Input: part model. Units: mm. Frame: model coordinates. A direction names the side the tool comes from. Coordinates: 2 decimals unless noted, no trailing zeros. Write each loop counter-clockwise with the first axis right and the second up, starting at its lowest first coordinate (ties: lowest second). Pieces come first, ordered by that corner, then holes. Notation, with made-up numbers: M -8,-38 L 4,-38 A23 cw 4,-20 Z; hole C -13.5,14.5 d4. An arc over 180 degrees is marked long. Use one line per item in the form item = value.
from build123d import *

# Parameters (mm, degrees)
BOSS_EXTRUDE1_DEPTH          = 30
CUT_EXTRUDE1_DEPTH           = 15
F_9_0_9_DIAMETER_HOLE1_D     = 9
F_9_0_9_DIAMETER_HOLE1_DEPTH = 10
F_9_0_9_DIAMETER_HOLE1_TIP   = 2.703872786
M8_TAPPED_HOLE1_D            = 6.8


with BuildPart() as part:
    # Sketch1 → Boss-Extrude1 (new body)
    with BuildSketch(Plane.XY):
        Polygon((0, 0), (0, 10), (17.5, 10), (17.5, 50), (42.5, 50), (42.5, 10), (60, 10), (60, 0), align=None)
    extrude(amount=BOSS_EXTRUDE1_DEPTH)

    # Sketch2 → Cut-Extrude1 (cut)
    with BuildSketch(Plane.XY.offset(30)):
        with BuildLine():
            Line((38.5, 50), (38.5, 35))
            ThreePointArc((38.5, 35), (30, 26.5), (21.5, 35))
            Line((21.5, 35), (21.5, 50))
            ThreePointArc((21.5, 50), (30, 58.5), (38.5, 50))
        make_face()
    extrude(amount=-CUT_EXTRUDE1_DEPTH, mode=Mode.SUBTRACT)

    # Ø9.0 (9) Diameter Hole1
    with Locations(Plane(origin=(7.5, 0, 15), x_dir=(-1, 0, 0), z_dir=(0, -1, 0))):
        with Locations((0, 0), (-45, 0)):
            Hole(F_9_0_9_DIAMETER_HOLE1_D / 2, depth=F_9_0_9_DIAMETER_HOLE1_DEPTH)
            with Locations((0, 0, -(F_9_0_9_DIAMETER_HOLE1_DEPTH + F_9_0_9_DIAMETER_HOLE1_TIP / 2))):  # 118° drill point
                Cone(0, F_9_0_9_DIAMETER_HOLE1_D / 2, F_9_0_9_DIAMETER_HOLE1_TIP, mode=Mode.SUBTRACT)

    # M8 Tapped Hole1 (through all)
    with Locations(Plane(origin=(30, 39, 0), x_dir=(-1, 0, 0), z_dir=(0, 0, -1))):
        with Locations((0, 0)):
            Hole(M8_TAPPED_HOLE1_D / 2)


solid = part.part
(1) Line query: probe 1 along Z at (x, y) = (7.5, 2.75); probe 2 along Y at (x, z) = (30, 10.5); probe 3 along X at (y, z) = (44, 20.75). Output: solid intervals per line, ascending.
Computed:
probe_1 = 0 to 10.5, 19.5 to 30
probe_2 = 0 to 35.6, 42.4 to 50
probe_3 = 17.5 to 21.5, 38.5 to 42.5
(2) Section query B-B on y = 39. Return the cut outline in (x, z).
Computed:
outline = M 17.5,0 L 26.6,0 L 26.6,15 L 21.5,15 L 21.5,30 L 17.5,30 Z; M 33.4,0 L 42.5,0 L 42.5,30 L 38.5,30 L 38.5,15 L 33.4,15 Z
(3) Section query A-A on x = 52.5. Return the cut outline in (y, z).
Computed:
outline = M 0,0 L 10,0 L 10,10.5 L 0,10.5 Z; M 0,19.5 L 10,19.5 L 10,30 L 0,30 Z
(4) Section query D-D on y = 8. Return the cut outline in (x, z), plus the area to 3 significant figures.
Computed:
outline = M 0,0 L 60,0 L 60,30 L 0,30 Z; hole C 7.5,15 d9; hole C 52.5,15 d9
area = 1,670 mm^2
(5) Section query C-C on z = 28.25. Return the cut outline in (x, y), plus the area to 3 significant figures.
Computed:
outline = M 0,0 L 60,0 L 60,10 L 42.5,10 L 42.5,50 L 38.5,50 L 38.5,35 A8.5 cw 21.5,35 L 21.5,50 L 17.5,50 L 17.5,10 L 0,10 Z
area = 1,230 mm^2
(6) Pull-direction query (X, two-part tool) for faces 4 (the flat face through (38.5, 43, 23)), 5 (the flat face through (13, 10, 15)), 6 (the flat face through (17.5, 30, 15)); classes: pulls with the +X half, pulls with the -X half, needs draft (parallel to the pull), parting line crosses it, or undercut.
Computed:
face_4 = undercut
face_5 = needs draft
face_6 = pulls with the -X half
(7) First-contact query: pin 1 Ø13.5 at (x, y) = (28.5, 42.5) entering from +Z; pin 2 Ø14.5 at (x, z) = (7.5, 15) entering from +Y; pin 3 Ø12 at (y, z) = (44.5, 22.5) entering from -X; pin 4 Ø3 at (x, y) = (29.5, 38.5) entering from -Z. Flat tips, straight axial feed; report the tip coordinate or a pass-through.
Computed:
pin_1 = 15
pin_2 = 10
pin_3 = 17.5
pin_4 = through
(8) Set-up query: faces 1 (the flat face through (21.5, 42, 23)), 2 (the cylindrical face through (31.828, 41.867, 7.605)), 3 (the flat face through (47, 10, 15)). Return all of +Z, -Z, +X, -X, +Y, -Y with unobstructed straight access to the full face (end or side cutting, diameter ignored); none if empty.
Computed:
face_1 = +Z, +Y
face_2 = +Z, -Z
face_3 = +Z, -Z, +X, +Y
